Read the model definition and answer for the solid it produces. Units are mm, in the model's axes. A direction names the side the tool comes from. Give positions to 0.01 mm unless a question says otherwise; leave off trailing zeros. Loops run counter-clockwise (first coordinate to the right, second up) from the corner with the lowest first, then second, coordinate; pieces in that order, holes last.
(1) Find section A-A, the plane z = 1.5. Write down the section's boundary in (x, y).
(2) Straight lines are drawn through the part: probe 1 along Y at (x, z) = (4, 5); probe 2 along Y at (x, z) = (-9, 9); probe 3 along X at (y, z) = (19.5, 11.75). For each, find the intervals that lie inside material, in ascending order.
(3) Find section D-D, the plane y = -4.5. Write down the section's boundary in (x, z).
(4) Determine the mould class of faces 1 (the face through (-15, 0, 6)), 2 (the face through (-10.4, 18.6, 3)), 3 (the face through (0, 0, 12)) for opening direction X: pulls with the +X half, pulls with the -X half, needs draft (parallel to the pull), parting line crosses it, or undercut.
(5) Find section C-C, the plane x = -9. Write down the section's boundary in (y, z).
(6) Which of the six approach directions +Z, -Z, +X, -X, +Y, -Y give full straight-line access (tool end or side, diameter ignored) to faces 4 (the face through (15, 0, 6)), 5 (the face through (1.6, 18.6, 3))?
(7) Each of these flat-tipped pins is pushed along its axis until it touches: P1, Ø2, axis at x = 2, y = 20, coming from the -Z side; P2, Ø2, axis at x = -9, y = 20, coming from the +Z side. Where does it stop, or does it pass through?
(8) Find section B-B, the plane y = -19.5. Write down the section's boundary in (x, z), then the cut area to 3 significant figures.
```python
from build123d import *

# Parameters (mm, degrees)
SKETCH_1_W                                         = 30
SKETCH_1_H                                         = 50
BOSS_EXTRUDE_1_DEPTH                               = 12
M6_TAPPED_HOLE_1_D                                 = 5
M3_SOCKET_HEAD_CAP_SCREW_COUNTERBORE_1_D           = 3.4
M3_SOCKET_HEAD_CAP_SCREW_COUNTERBORE_1_CBORE_D     = 6.5
M3_SOCKET_HEAD_CAP_SCREW_COUNTERBORE_1_CBORE_DEPTH = 3
LINEAR_PATTERN_1_COUNT                             = 2
LINEAR_PATTERN_1_PITCH                             = 12


with BuildPart() as part:
    # Sketch 1 → Boss-Extrude 1 (new body)
    with BuildSketch(Plane.XY):
        Rectangle(SKETCH_1_W, SKETCH_1_H)
    extrude(amount=BOSS_EXTRUDE_1_DEPTH)

    # M6 Tapped Hole 1 (through all)
    with Locations(Plane(origin=(0, 0, 0), x_dir=(-1, 0, 0), z_dir=(0, 0, -1))):
        with Locations((7.5, -4), (-2.5, -18)):
            Hole(M6_TAPPED_HOLE_1_D / 2)

    # M3 Socket Head Cap Screw Counterbore 1 (through all)
    with Locations(Plane(origin=(0, 0, 0), x_dir=(-1, 0, 0), z_dir=(0, 0, -1))):
        with Locations((9, 20)):
            m3_socket_head_cap_screw_counterbore_1 = CounterBoreHole(M3_SOCKET_HEAD_CAP_SCREW_COUNTERBORE_1_D / 2, M3_SOCKET_HEAD_CAP_SCREW_COUNTERBORE_1_CBORE_D / 2, M3_SOCKET_HEAD_CAP_SCREW_COUNTERBORE_1_CBORE_DEPTH)

    # Linear Pattern 1: M3 Socket Head Cap Screw Counterbore 1 ×2
    with Locations(*[(i * LINEAR_PATTERN_1_PITCH, 0, 0) for i in range(1, LINEAR_PATTERN_1_COUNT)]):
        add(m3_socket_head_cap_screw_counterbore_1, mode=Mode.SUBTRACT)


solid = part.part
```
Entries:
1. outline: (-15, -25) - (15, -25) - (15, 25) - (-15, 25) - close; hole circle Ø6.5 at (-9, 20); hole circle Ø5 at (-7.5, -4); hole circle Ø6.5 at (3, 20); hole circle Ø5 at (2.5, -18)
2. probe 1: y = -25 to -20, -16 to 18.63, 21.37 to 25
2. probe 2: y = -25 to -6, -2 to 18.3, 21.7 to 25
2. probe 3: x = -15 to -10.62, -7.38 to 1.38, 4.62 to 15
3. outline: (-15, 0) - (-9.95, 0) - (-9.95, 12) - (-15, 12) - close; (-5.05, 0) - (15, 0) - (15, 12) - (-5.05, 12) - close
4. face 1: pulls with the -X half
4. face 2: undercut
4. face 3: needs draft
5. outline: (-25, 0) - (-6, 0) - (-6, 12) - (-25, 12) - close; (-2, 0) - (16.75, 0) - (16.75, 3) - (18.3, 3) - (18.3, 12) - (-2, 12) - close; (21.7, 3) - (23.25, 3) - (23.25, 0) - (25, 0) - (25, 12) - (21.7, 12) - close
6. face 4: +Z, -Z, +X, +Y, -Y
6. face 5: -Z
7. P1: stops at z = 3
7. P2: passes through
8. outline: (-15, 0) - (0.5, 0) - (0.5, 12) - (-15, 12) - close; (4.5, 0) - (15, 0) - (15, 12) - (4.5, 12) - close
8. area: 312 mm2
